Geometry check sheet. Reference: the model listing, model coordinates, mm. Round coordinates to 2 decimals unless told otherwise and drop trailing zeros.
```python
from build123d import *

# Parameters (mm, degrees)
SKETCH_1_W      = 78.5
SKETCH_1_H      = 53.5
EXTRUDE_1_DEPTH = 14
FILLET_1_R      = 6


with BuildPart() as part:
    # 草图1 → 凸台-拉伸1 (new body)
    with BuildSketch(Plane.XY):
        with Locations((39.25, 26.75)):
            Rectangle(SKETCH_1_W, SKETCH_1_H)
    extrude(amount=EXTRUDE_1_DEPTH)

    # 圆角1
    fillet_1_edges = [part.edges().sort_by_distance(p)[0] for p in [
        (0, 53.5, 7),
        (78.5, 53.5, 7),
        (78.5, 0, 7),
        (0, 0, 7),
    ]]
    fillet(fillet_1_edges, radius=FILLET_1_R)


solid = part.part
```
1) Mould release check, pull along Z, two halves, no side actions. Record for faces 1 (the face through (39, 27, 14)), 2 (the face through (76.789, 51.696, 7.098)), 3 (the face through (39, 27, 0)): +Z half, -Z half, draft (parallel to the pull), parting line (faces both ways), or undercut.
Report:
face 1: +Z half
face 2: draft
face 3: -Z half
2) Gauge pin test, flat end, axial feed: pin 1 (3 mm diameter, centred on x = 62, y = 44, fed in from -Z). Record the tip position at first contact, or that the pin passes through.
Report:
pin 1: stops at z = 0
3) Scan line: line 1 along Y through (x, z) = (4, 2.5). Record every from-to range of solid material in increasing order.
Report:
line 1: y = 0.34 to 53.16
